Here's the drawing with two shaded views (mm, measured from the low corner). I have some questions. Round coordinates to 2 decimals unless told otherwise and drop trailing zeros. Write each loop counter-clockwise with the first axis right and the second up, starting at its lowest first coordinate (ties: lowest second). Pieces come first, ordered by that corner, then holes. Notation, with made-up numbers: M 41,86.5 L 78,86.5 A29 cw 78,119.5 Z; hole C 5.5,48.25 d10. An arc over 180 degrees is marked long. Write item = value, one per line. Start each with the question number.
(1) I want a section at D-D (x = 28.5). List the corners of the cut face in (y, z) for me.
(2) I want a section at C-C (z = 1.35). List the corners of the cut face in (x, y) for me.
(3) I need wall thicknesses on line 1 along Y through (x, z) = (7, 1.1); line 2 along Y through (x, z) = (28.5, 0.45). Which ranges of each line are inside material? Lowest first, please.
(4) I want a section at A-A (x = 7). List the corners of the cut face in (y, z) for me.
(5) I want a section at B-B (y = 7.5). List the corners of the cut face in (x, z) for me.
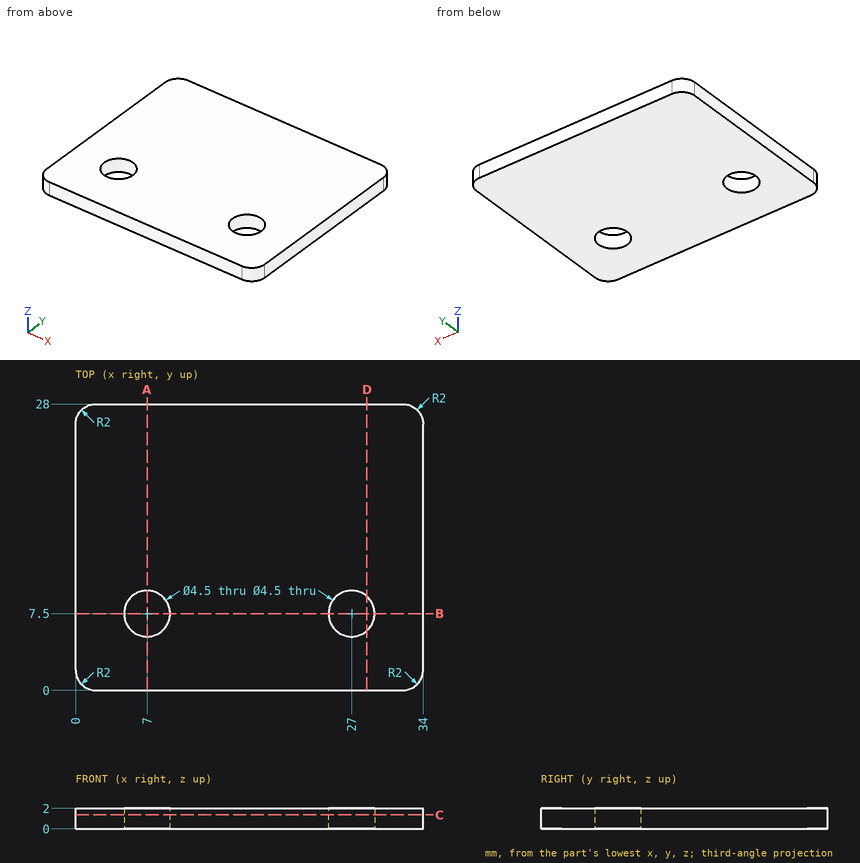
Returned:
q1.outline = M 0,0 L 5.82,0 L 5.82,2 L 0,2 Z; M 9.18,0 L 28,0 L 28,2 L 9.18,2 Z
q2.outline = M 0,2 A2 ccw 2,0 L 32,0 A2 ccw 34,2 L 34,26 A2 ccw 32,28 L 2,28 A2 ccw 0,26 Z; hole C 7,7.5 d4.5; hole C 27,7.5 d4.5
q3.line_1 = 0 to 5.25, 9.75 to 28
q3.line_2 = 0 to 5.82, 9.18 to 28
q4.outline = M 0,0 L 5.25,0 L 5.25,2 L 0,2 Z; M 9.75,0 L 28,0 L 28,2 L 9.75,2 Z
q5.outline = M 0,0 L 4.75,0 L 4.75,2 L 0,2 Z; M 9.25,0 L 24.75,0 L 24.75,2 L 9.25,2 Z; M 29.25,0 L 34,0 L 34,2 L 29.25,2 Z
